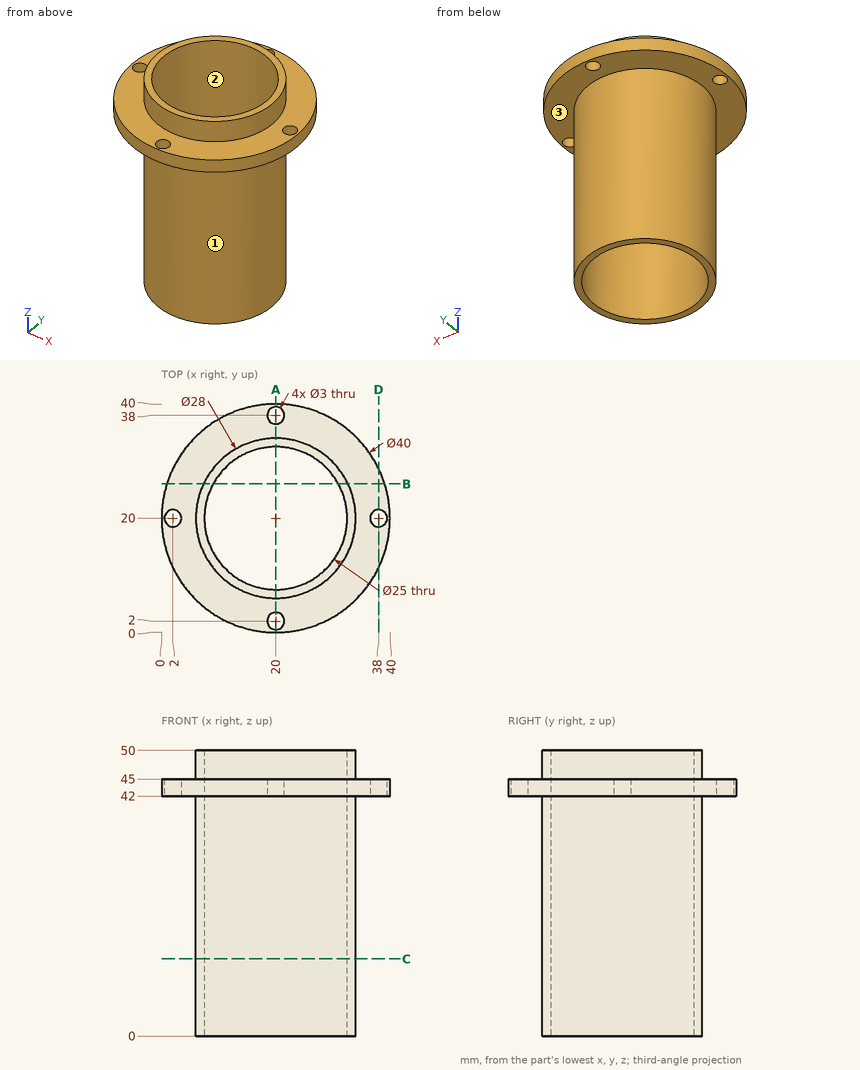
Job drawing, mm, ordinate dimensions from the low corner. One solid piece. Give positions to 0.01 mm unless a question says otherwise; leave off trailing zeros. Order: outer loops, then holes, each group sorted by start corner. A loop starts at its lowest first (then second) coordinate and runs counter-clockwise, first axis right, second up. Notation, with made-up numbers: M 37.5,54 L 92.5,54 A11 ccw 92.5,69 Z; hole C 66,17 d9. An arc over 180 degrees is marked long. Put each result on its own line as item: value. Start each with the question number.
(1) Pin check, flat tips, straight feed: pin 1 Ø6 at (x, z) = (27, 25.5) entering from +Y; pin 2 Ø5 at (x, y) = (11, 26.5) entering from -Z; pin 3 Ø3 at (x, z) = (14.5, 44) entering from -Y; pin 4 Ø4 at (x, z) = (21.5, 26.5) entering from +Y. Stop position of each tip, or through.
(2) Drill centre lines: L1, parallel to Y at x = 20, z = 42.65; L2, parallel to Y at x = 20, z = 30; L3, parallel to X at y = 15, z = 23. Where is each one in solid material? Low to high. Write a range as [from, to].
(3) Pull direction Y, two halves, no side cores. Call the marked faces 1, 2 and 3: released by +Y, released by -Y, zero draft, split by the parting line, or undercut.
(4) Band-saw the part on A-A on x = 20. Give the cut face in (y, z), then the cut area to 3 significant figures.
(5) Band-saw the part on B-B on y = 26. Give the cut face in (x, z).
(6) Band-saw the part on D-D on x = 38. Give the cut face in (y, z), then the cut area to 3 significant figures.
(7) Band-saw the part on C-C on z = 13.5. Give the cut face in (x, y), then the cut area to 3 significant figures.
Results below:
1. pin 1: stops at y = 33.42
1. pin 2: stops at z = 0
1. pin 3: stops at y = 0.4
1. pin 4: stops at y = 34
2. L1: y = [0, 0.5], [3.5, 7.5], [32.5, 36.5], [39.5, 40]
2. L2: y = [6, 7.5], [32.5, 34]
2. L3: x = [6.92, 8.54], [31.46, 33.08]
3. face 1: split by the parting line
3. face 2: undercut
3. face 3: zero draft
4. outline: M 0,42 L 0.5,42 L 0.5,45 L 0,45 Z; M 3.5,42 L 6,42 L 6,0 L 7.5,0 L 7.5,50 L 6,50 L 6,45 L 3.5,45 Z; M 32.5,0 L 34,0 L 34,42 L 36.5,42 L 36.5,45 L 34,45 L 34,50 L 32.5,50 Z; M 39.5,42 L 40,42 L 40,45 L 39.5,45 Z
4. area: 168 mm2
5. outline: M 0.92,42 L 7.35,42 L 7.35,0 L 9.03,0 L 9.03,50 L 7.35,50 L 7.35,45 L 0.92,45 Z; M 30.97,0 L 32.65,0 L 32.65,42 L 39.08,42 L 39.08,45 L 32.65,45 L 32.65,50 L 30.97,50 Z
6. outline: M 11.28,42 L 18.5,42 L 18.5,45 L 11.28,45 Z; M 21.5,42 L 28.72,42 L 28.72,45 L 21.5,45 Z
6. area: 43.3 mm2
7. outline: C 20,20 d28; hole C 20,20 d25
7. area: 125 mm2
